For this review, take the finished solid that the model builds, in its own axes (mm). Face numbers are marked on the shaded views. Give positions to 0.01 mm unless a question says otherwise; leave off trailing zeros. Order: outer loops, then holes, each group sorted by start corner. A loop starts at its lowest first (then second) coordinate and runs counter-clockwise, first axis right, second up. Notation, with made-up numbers: (-25.5, -38.5) -> (-2.5, -38.5) arc R12 cw to (-2.5, -23.5) -> close; hole circle Ø1 at (-4.5, 64). An arc over 180 degrees is marked (long way). One line per item, written item: value. Start each with the question number.
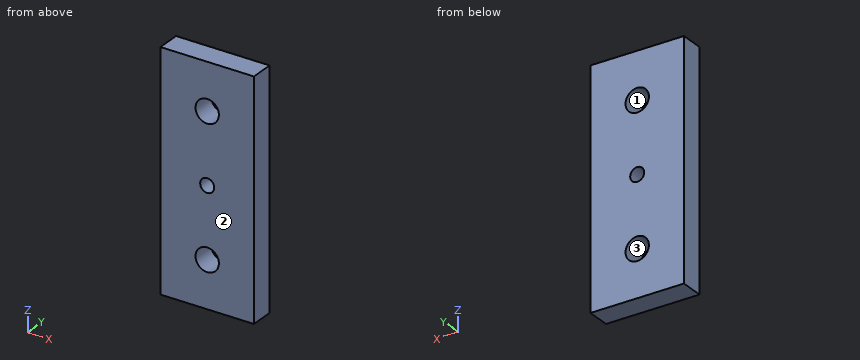
from build123d import *

# Parameters (mm, degrees)
SKETCH1_W           = 40
SKETCH1_H           = 100
SKETCH1_R           = 5
SKETCH1_R_2         = 3
BOSS_EXTRUDE1_DEPTH = 10


with BuildPart() as part:
    # Sketch1 → Boss-Extrude1 (new body)
    with BuildSketch(Plane(origin=(0, 0, 0), x_dir=(1, 0, 0), z_dir=(0, 1, 0))):
        Rectangle(SKETCH1_W, SKETCH1_H)
        with Locations(Location((0, 30, 0), (0, 0, 270))):
            Circle(SKETCH1_R, mode=Mode.SUBTRACT)
        with Locations(Location((0, -30, 0), (0, 0, 270))):
            Circle(SKETCH1_R, mode=Mode.SUBTRACT)
        with Locations(Location((0, 0, 0), (0, 0, 270))):
            Circle(SKETCH1_R_2, mode=Mode.SUBTRACT)
    extrude(amount=BOSS_EXTRUDE1_DEPTH)


solid = part.part
Q1. Take a section at B-B (y = 7). State the section outline as (x, z) points.
Q2. For line 1 along X through (y, z) = (2.25, 30); line 2 along X through (y, z) = (7.25, 0); line 3 along Z through (x, y) = (0.5, 2), list the stretches that pass through material, from the lowest coordinate up.
Q3. Take a section at A-A (z = -33). State the section outline as (x, y) points.
Q4. Mouldability with a two-part tool opening along Z and no side actions: class the marked faces 1, 2 and 3 as pulls with the +Z half, pulls with the -Z half, needs draft (parallel to the pull), parting line crosses it, or undercut.
Q5. Take a section at C-C (x = 0). State the section outline as (y, z) points.
Q6. For pin 1 Ø8 at (x, z) = (0, -30) entering from +Y, flat-tipped, find the tip position at first contact; note if it passes through.
Q7. Take a section at D-D (z = 0). State the section outline as (x, y) points, and give its area (3 significant figures).
Answers below:
1. outline: (-20, -50) -> (20, -50) -> (20, 50) -> (-20, 50) -> close; hole circle Ø10 at (0, -30); hole circle Ø10 at (0, 30); hole circle Ø6 at (0, 0)
2. line 1: x = -20 to -5, 5 to 20
2. line 2: x = -20 to -3, 3 to 20
2. line 3: z = -50 to -34.97, -25.03 to -2.96, 2.96 to 25.03, 34.97 to 50
3. outline: (-20, 0) -> (-4, 0) -> (-4, 10) -> (-20, 10) -> close; (4, 0) -> (20, 0) -> (20, 10) -> (4, 10) -> close
4. face 1: undercut
4. face 2: needs draft
4. face 3: undercut
5. outline: (0, -50) -> (10, -50) -> (10, -35) -> (0, -35) -> close; (0, -25) -> (10, -25) -> (10, -3) -> (0, -3) -> close; (0, 3) -> (10, 3) -> (10, 25) -> (0, 25) -> close; (0, 35) -> (10, 35) -> (10, 50) -> (0, 50) -> close
6. pin 1: passes through
7. outline: (-20, 0) -> (-3, 0) -> (-3, 10) -> (-20, 10) -> close; (3, 0) -> (20, 0) -> (20, 10) -> (3, 10) -> close
7. area: 340 mm²
